Work out the finished part from the listing and answer in its coordinate system (mm). Face numbers are marked on the shaded views. Round coordinates to 2 decimals unless told otherwise and drop trailing zeros. Loops run counter-clockwise (first coordinate to the right, second up) from the corner with the lowest first, then second, coordinate; pieces in that order, holes last. Notation, with made-up numbers: (27, 87.5) -> (86, 87.5) arc R15 ccw to (86, 107.5) -> close; hole circle Ø1 at (40, 47.25). An arc over 180 degrees is marked (long way). Use one line per item in the form item = value.
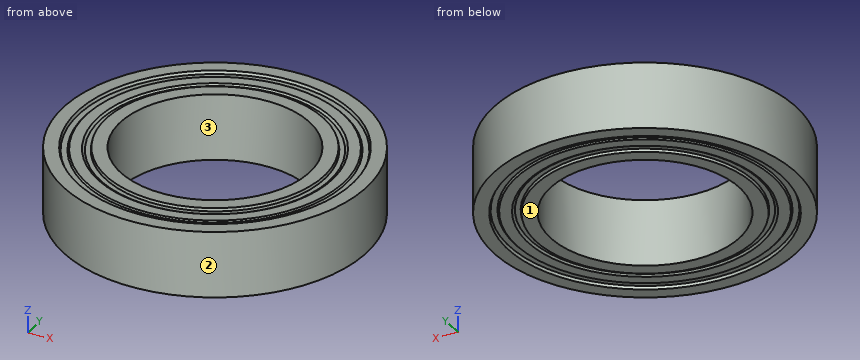
```python
from build123d import *

# Parameters (mm, degrees)
SKETCH1_R           = 16
SKETCH1_R_2         = 10
BOSS_EXTRUDE1_DEPTH = 7


with BuildPart() as part:
    # Sketch1 → Boss-Extrude1 (new body)
    with BuildSketch(Plane.XY):
        Circle(SKETCH1_R)
        Circle(SKETCH1_R_2, mode=Mode.SUBTRACT)
    extrude(amount=BOSS_EXTRUDE1_DEPTH)

    # Sketch3 → Cut-Revolve1 (revolve, cut)
    with BuildSketch(Plane(origin=(0, 0, 0), x_dir=(1, 0, 0), z_dir=(0, 1, 0)), mode=Mode.PRIVATE) as cut_revolve1_sk:
        Polygon((11.5, -7), (11.567254185, -6.694573787), (12.105287665, -6.694573787), (12.374680794, -6.847286894), (13.574680794, -6.847286894), (13.7273939, -6.694573787), (14.365955247, -6.694573787), (14.5, -7), align=None)
    cut_revolve1 = revolve(cut_revolve1_sk.sketch.rotate(Axis((0, 0, 0), (0, 0, 1)), 180), axis=Axis((0, 0, 0), (0, 0, 1)), mode=Mode.SUBTRACT)

    # Mirror1: Cut-Revolve1 across plane
    add(cut_revolve1.mirror(Plane.XY.offset(3.5)), mode=Mode.SUBTRACT)


solid = part.part
```
(1) For a pull along Y with two mould halves and no side action, classify the marked faces 1, 2 and 3 as +Y half, -Y half, draft (parallel to the pull), parting line (faces both ways), or undercut.
Completed:
face_1 = draft
face_2 = parting line
face_3 = undercut
(2) Find section A-A, the plane z = 5.75. Write down the section's boundary in (x, y).
Completed:
outline = circle Ø32 at (0, 0); hole circle Ø20 at (0, 0)
(3) Given P1, Ø4, axis at x = 11.5, z = 1, coming from the -Y side, flat-ended and moving along its own axis, determine where the tip first touches the part or whether it passes through.
Completed:
P1 = -12.87
(4) Consider L1, parallel to Y at x = 0, z = 5; L2, parallel to X at y = 3, z = 2.5; L3, parallel to X at y = -6, z = 6. Determine where each line is inside the solid, lowest interval first.
Completed:
L1 = -16 to -10, 10 to 16
L2 = -15.72 to -9.54, 9.54 to 15.72
L3 = -14.83 to -8, 8 to 14.83
